from build123d import *

# Parameters (mm, degrees)
SKETCH_1_R      = 6
EXTRUDE_1_DEPTH = 13.5
CHAMFER_1_SIZE  = 0.5
SKETCH_2_R      = 2.5
EXTRUDE_2_DEPTH = 12
CHAMFER_2_SIZE  = 0.2
SKETCH_3_R      = 7.5
EXTRUDE_3_DEPTH = 21
CHAMFER_3_SIZE  = 0.2


with BuildPart() as part:
    # 草图1 → 凸台-拉伸1 (new, symmetric)
    with BuildSketch(Plane.XY):
        Circle(SKETCH_1_R)
    extrude(amount=EXTRUDE_1_DEPTH, both=True)

    # 倒角1
    chamfer_1_edges = [part.edges().sort_by_distance(p)[0] for p in [
        (-6, 0, -13.5),
        (-6, 0, 13.5),
    ]]
    chamfer(chamfer_1_edges, length=CHAMFER_1_SIZE)

    # 草图2 → 凸台-拉伸2 (add)
    with BuildSketch(Plane.XY.offset(13.5)):
        Circle(SKETCH_2_R)
    extrude(amount=EXTRUDE_2_DEPTH)

    # 倒角2
    chamfer_2_edges = [part.edges().sort_by_distance(p)[0] for p in [
        (-2.5, 0, 25.5),
    ]]
    chamfer(chamfer_2_edges, length=CHAMFER_2_SIZE)

    # 草图3 → 凸台-拉伸3 (add)
    with BuildSketch(Plane.XY.offset(13.5)):
        Circle(SKETCH_3_R)
    extrude(amount=-EXTRUDE_3_DEPTH)

    # 倒角3
    chamfer_3_edges = [part.edges().sort_by_distance(p)[0] for p in [
        (-7.5, 0, 13.5),
        (-7.5, 0, -7.5),
    ]]
    chamfer(chamfer_3_edges, length=CHAMFER_3_SIZE)


solid = part.part
Read the model definition and answer for the solid it produces. Units are mm, in the model's axes. A direction names the side the tool comes from. Give positions to 0.01 mm unless a question says otherwise; leave off trailing zeros. Loops run counter-clockwise (first coordinate to the right, second up) from the corner with the lowest first, then second, coordinate; pieces in that order, holes last. Notation, with made-up numbers: (44.5, 41) -> (49.5, 41) arc R27 cw to (49.5, 65) -> close; hole circle Ø1 at (1, -22). An arc over 180 degrees is marked (long way). Answer as CSV lines item,"result".
Item 1: Find section D-D on z = -10.5. Give the vertices of the cut face in (x, y), plus the area to 3 significant figures.
Returned:
outline,"circle Ø12 at (0, 0)"
area,"113 mm²"
Item 2: Consider line 1 (Z direction, x = -6.5, y = -1.25); line 2 (Z direction, x = 1.5, y = -5); line 3 (X direction, y = -1.75, z = 10). Determine where each line is inside the solid, lowest interval first. Write a range as [from, to].
Returned:
line 1,"z = [-7.5, 13.5]"
line 2,"z = [-13.5, 13.5]"
line 3,"x = [-7.29, 7.29]"
Item 3: Find section A-A on y = 0. Give the vertices of the cut face in (x, z), plus the area to 3 significant figures.
Returned:
outline,"(-7.5, -7.3) -> (-7.3, -7.5) -> (-6, -7.5) -> (-6, -13) -> (-5.5, -13.5) -> (5.5, -13.5) -> (6, -13) -> (6, -7.5) -> (7.3, -7.5) -> (7.5, -7.3) -> (7.5, 13.3) -> (7.3, 13.5) -> (2.5, 13.5) -> (2.5, 25.3) -> (2.3, 25.5) -> (-2.3, 25.5) -> (-2.5, 25.3) -> (-2.5, 13.5) -> (-7.3, 13.5) -> (-7.5, 13.3) -> close"
area,"447 mm²"
Item 4: For faces 1 (the face through (-2, -6, -7.5)), 2 (the face through (0, 0, 25.5)), 3 (the face through (-0.54, -2.44, 19.32)), determine the directions among +Z, -Z, +X, -X, +Y, -Y from which every point of the face is accessible in a straight line to the end or side of a thin tool.
Returned:
face 1,"-Z"
face 2,"+Z, +X, -X, +Y, -Y"
face 3,"+Z"
Item 5: Each of these flat-tipped pins is pushed along its axis until it touches: pin 1 (4 mm diameter, centred on x = -2, z = 9.5, fed in from +Y); pin 2 (2 mm diameter, centred on y = 3, z = 15, fed in from +X); pin 3 (1 mm diameter, centred on x = 2.5, z = -6.5, fed in from +Y); pin 4 (1.5 mm diameter, centred on y = 1.5, z = 4.5, fed in from -X). Where does it stop, or does it pass through?
Returned:
pin 1,"stops at y = 7.5"
pin 2,"stops at x = 1.5"
pin 3,"stops at y = 7.23"
pin 4,"stops at x = -7.46"
Item 6: Find section C-C on z = -1. Give the vertices of the cut face in (x, y).
Returned:
outline,"circle Ø15 at (0, 0)"
